Read the model definition and answer for the solid it produces. Units are mm, in the model's axes. A direction names the side the tool comes from. Coordinates: 2 decimals unless noted, no trailing zeros. Write each loop counter-clockwise with the first axis right and the second up, starting at its lowest first coordinate (ties: lowest second). Pieces come first, ordered by that corner, then holes. Notation, with made-up numbers: (28.25, 47) - (83.25, 47) arc R34 cw to (83.25, 86) - close; hole circle Ø5 at (29.5, -35). An arc over 180 degrees is marked (long way). Return JSON: item names as keys, results as strings.
```python
from build123d import *

# Parameters (mm, degrees)
SKETCH1_W           = 20
SKETCH1_H           = 11.2
BOSS_EXTRUDE1_DEPTH = 30
SKETCH2_R           = 3
BOSS_EXTRUDE2_DEPTH = 1.2
FILLET1_R           = 2
SKETCH3_R           = 0.6
BOSS_EXTRUDE3_DEPTH = 1


with BuildPart() as part:
    # Sketch1 → Boss-Extrude1 (new body)
    with BuildSketch(Plane(origin=(0, 0, 0), x_dir=(1, 0, 0), z_dir=(0, 1, 0))):
        Rectangle(SKETCH1_W, SKETCH1_H)
    extrude(amount=BOSS_EXTRUDE1_DEPTH)

    # Sketch2 → Boss-Extrude2 (add)
    with BuildSketch(Plane.XY.offset(5.6)):
        with BuildLine():
            Line((-1.5, 55.197386366), (-7.5, 30))
            Line((-7.5, 30), (7.5, 30))
            Line((7.5, 30), (1.5, 55.197386366))
            Line((1.5, 55.197386366), (1.5, 55.727386366))
            ThreePointArc((1.5, 55.727386366), (0, 62.6), (-1.5, 55.727386366))
            Line((-1.5, 55.727386366), (-1.5, 55.197386366))
        make_face()
        with Locations((0, 59)):
            Circle(SKETCH2_R, mode=Mode.SUBTRACT)
    extrude(amount=-BOSS_EXTRUDE2_DEPTH)

    # Fillet1
    fillet1_edges = [part.edges().sort_by_distance(p)[0] for p in [
        (-10, 15, -5.6),
        (10, 15, -5.6),
    ]]
    fillet(fillet1_edges, radius=FILLET1_R)

    # Sketch3 → Boss-Extrude3 (add)
    # profile 1 of 2: a face of its own
    with BuildSketch(Plane.XZ):
        with BuildLine():
            Line((6.5, -5.6), (4, -5.6))
            Line((4, -5.6), (4, -6.85))
            ThreePointArc((4, -6.85), (5.25, -8.1), (6.5, -6.85))
            Line((6.5, -6.85), (6.5, -5.6))
        make_face()
        with Locations(Location((5.25, -6.85, 0), (0, 0, 90))):
            Circle(SKETCH3_R, mode=Mode.SUBTRACT)
    # profile 2 of 2: a face of its own
    with BuildSketch(Plane.XZ):
        with BuildLine():
            Line((-6.5, -5.6), (-4, -5.6))
            Line((-4, -5.6), (-4, -6.85))
            ThreePointArc((-4, -6.85), (-5.25, -8.1), (-6.5, -6.85))
            Line((-6.5, -6.85), (-6.5, -5.6))
        make_face()
        with Locations(Location((-5.25, -6.85, 0), (0, 0, 270))):
            Circle(SKETCH3_R, mode=Mode.SUBTRACT)
    extrude(amount=-BOSS_EXTRUDE3_DEPTH)


solid = part.part
```
(1) Straight lines are drawn through the part: line 1 (X direction, y = 0.45, z = -6.85); line 2 (Z direction, x = 2.5, y = 57); line 3 (Y direction, x = -8.25, z = -3.75). For each, find the intervals that lie inside material, in ascending order. Write a range as from..to.
Answer:
{"line 1": "-6.5..-5.85, -4.65..-4, 4..4.65, 5.85..6.5", "line 2": "4.4..5.6", "line 3": "0..30"}
(2) Determine the mould class of faces 1 (the face through (-5.2, 0.5, -8.1)), 2 (the face through (0, 0, 0)), 3 (the face through (0.1, 62.6, 5)) for opening direction Y: +Y half, -Y half, draft (parallel to the pull), parting line (faces both ways), or undercut.
Answer:
{"face 1": "draft", "face 2": "-Y half", "face 3": "undercut"}
(3) A cutting plane is placed at A-A (y = 59). Determine the outline of the cut face in (x, z), and give its area (3 significant figures).
Answer:
{"outline": "(-3.6, 4.4) - (-3, 4.4) - (-3, 5.6) - (-3.6, 5.6) - close; (3, 4.4) - (3.6, 4.4) - (3.6, 5.6) - (3, 5.6) - close", "area": "1.44 mm²"}
(4) A cutting plane is placed at D-D (x = 5.25). Determine the outline of the cut face in (y, z).
Answer:
{"outline": "(0, -8.1) - (1, -8.1) - (1, -7.45) - (0, -7.45) - close; (0, -6.25) - (1, -6.25) - (1, -5.6) - (30, -5.6) - (30, 4.4) - (39.45, 4.4) - (39.45, 5.6) - (0, 5.6) - close"}
(5) A cutting plane is placed at C-C (z = -2). Determine the outline of the cut face in (x, y).
Answer:
{"outline": "(-10, 0) - (10, 0) - (10, 30) - (-10, 30) - close"}
(6) Flat-ended cylindrical pins translate along their axes: P1, Ø2, axis at x = 4.5, z = -6.5, coming from the +Y side; P2, Ø1.5, axis at y = 50, z = 3.5, coming from the -X side; P3, Ø10, axis at x = -5.5, y = 22, coming from the -Z side; P4, Ø0.5, axis at y = 0.5, z = -6, coming from the -X side. Find the tip coordinate at first contact, or state that the pin passes through.
Answer:
{"P1": "y = 30", "P2": "through", "P3": "z = -5.6", "P4": "x = -6.5"}
(7) Which of the six approach directions +Z, -Z, +X, -X, +Y, -Y give full straight-line access (tool end or side, diameter ignored) to faces 4 (the face through (0, 39, 4.4)), 5 (the face through (-4.458, 42.775, 5.008)), 6 (the face through (0, 24, 5.6))?
Answer:
{"face 4": "-Z, +X, -X, +Y", "face 5": "+Z, -Z, -X", "face 6": "+Z, +X, -X, +Y, -Y"}
(8) A cutting plane is placed at B-B (x = 0). Determine the outline of the cut face in (y, z).
Answer:
{"outline": "(0, -5.6) - (30, -5.6) - (30, 4.4) - (56, 4.4) - (56, 5.6) - (0, 5.6) - close; (62, 4.4) - (62.6, 4.4) - (62.6, 5.6) - (62, 5.6) - close"}
